Source: CAD feature listing. Evaluate the final solid. Frame: model axes, mm. A direction names the side the tool comes from. Round coordinates to 2 decimals unless told otherwise and drop trailing zeros. Order: outer loops, then holes, each group sorted by start corner. A loop starts at its lowest first (then second) coordinate and runs counter-clockwise, first axis right, second up. Notation, with made-up numbers: (-17.75, 29) - (32.25, 29) arc R19 ccw to (32.25, 45) - close; hole circle Ø10 at (-15, 17.5). An arc over 180 degrees is marked (long way). Put each result on its own line as item: value. Start each with the question number.
1) Line query: probe 1 along X at (y, z) = (0, 6.45); probe 2 along Y at (x, z) = (0, -21.65). Output: solid intervals per line, ascending. Write a range as [from, to].
2) Access query for faces 1 (the face through (-4.74, 2.79, 4.89)), 2 (the face through (0, 0, 5.8)), 3 (the face through (0, 0, 10.6)). Directions: +Z, -Z, +X, -X, +Y, -Y. A direction counts if a zero-diameter tool reaches every point of the face in a straight line with its end or side. Return the directions, or none.
3) Section C-C on z = 1. Output: boundary loops of the cut face in (x, y).
4) Section A-A on z = -21. Output: boundary loops of the cut face in (x, y), then the cut area to 3 significant figures.
5) Section D-D on y = -4.5. Output: boundary loops of the cut face in (x, z), then the cut area to 3 significant figures.
6) Contact query for flat-ended pins moving along their axis: P1, Ø2.5, axis at x = 0, y = 0, coming from the -Z side; P2, Ø5, axis at y = 3, z = -11.5, coming from the +X side; P3, Ø8, axis at x = 4.5, z = -7, coming from the +Y side; P4, Ø3.5, axis at x = 0.5, y = 0.5, coming from the +Z side. Output: stop coordinate, or through.
7) Section B-B on x = -5.5. Output: boundary loops of the cut face in (y, z), then the cut area to 3 significant figures.
8) Mould query, pull axis X, two halves, no side actions, for faces 4 (the face through (0, -5.5, 5)), 5 (the face through (0, 0, 7.3)), 6 (the face through (1.062, -4.783, -9.86)), 7 (the face through (-1.825, -1.4, 6.54)). Classes: +X half, -X half, draft (parallel to the pull), parting line (faces both ways), or undercut.
```python
from build123d import *

# Parameters (mm, degrees)
BOSS_EXTRUDE1_DEPTH = 4
BOSS_EXTRUDE2_DEPTH = 1.8
SKETCH3_R           = 2.65
SKETCH3_R_2         = 2.3
BOSS_EXTRUDE3_DEPTH = 5.8
BOSS_EXTRUDE4_START = -1
SKETCH4_R           = 3.15
BOSS_EXTRUDE4_DEPTH = 3.3
SKETCH5_R           = 4.9
BOSS_EXTRUDE5_DEPTH = 20
SKETCH6_R           = 3.15
SKETCH6_R_2         = 2.25
BOSS_EXTRUDE6_DEPTH = 6


with BuildPart() as part:
    # Sketch1 → Boss-Extrude1 (new body)
    with BuildSketch(Plane.XY):
        Polygon((8.082903769, 0), (4.041451884, 7), (-4.041451884, 7), (-8.082903769, 0), (-4.041451884, -7), (4.041451884, -7), align=None)
    extrude(amount=BOSS_EXTRUDE1_DEPTH)

    # Sketch2 → Boss-Extrude2 (add)
    with BuildSketch(Plane.XY.offset(4)):
        Polygon((6.350852961, 0), (3.175426481, 5.5), (-3.175426481, 5.5), (-6.350852961, 0), (-3.175426481, -5.5), (3.175426481, -5.5), align=None)
    extrude(amount=BOSS_EXTRUDE2_DEPTH)

    # Sketch3 → Boss-Extrude3 (add)
    with BuildSketch(Plane.XY.offset(5.8)):
        Circle(SKETCH3_R)
        Circle(SKETCH3_R_2, mode=Mode.SUBTRACT)
    extrude(amount=BOSS_EXTRUDE3_DEPTH)

    # Sketch4 → Boss-Extrude4 (add)
    with BuildSketch(Plane.XY.offset(11.6).offset(BOSS_EXTRUDE4_START)):
        Circle(SKETCH4_R)
    extrude(amount=-BOSS_EXTRUDE4_DEPTH)

    # Sketch5 → Boss-Extrude5 (add)
    with BuildSketch(Plane(origin=(0, 0, 0), x_dir=(-1, 0, 0), z_dir=(0, 0, -1))):
        Circle(SKETCH5_R)
    extrude(amount=BOSS_EXTRUDE5_DEPTH)

    # Sketch6 → Boss-Extrude6 (add)
    with BuildSketch(Plane(origin=(0, 0, -20), x_dir=(-1, 0, 0), z_dir=(0, 0, -1))):
        with Locations(Location((0, 0, 0), (0, 0, 180))):
            Circle(SKETCH6_R)
        Circle(SKETCH6_R_2, mode=Mode.SUBTRACT)
    extrude(amount=BOSS_EXTRUDE6_DEPTH)


solid = part.part
```
Answer sheet:
1. probe 1: [-2.65, -2.3], [2.3, 2.65]
1. probe 2: [-3.15, -2.25], [2.25, 3.15]
2. face 1: +Z, -X, +Y
2. face 2: none
2. face 3: +Z
3. outline: (-8.08, 0) - (-4.04, -7) - (4.04, -7) - (8.08, 0) - (4.04, 7) - (-4.04, 7) - close
4. outline: circle Ø6.3 at (0, 0); hole circle Ø4.5 at (0, 0)
4. area: 15.3 mm^2
5. outline: (-5.48, 0) - (-1.94, 0) - (-1.94, -20) - (1.94, -20) - (1.94, 0) - (5.48, 0) - (5.48, 4) - (3.75, 4) - (3.75, 5.8) - (-3.75, 5.8) - (-3.75, 4) - (-5.48, 4) - close
5. area: 135 mm^2
6. P1: z = -20
6. P2: x = 4.87
6. P3: y = 4.87
6. P4: z = 11.6
7. outline: (-4.47, 0) - (4.47, 0) - (4.47, 4) - (1.47, 4) - (1.47, 5.8) - (-1.47, 5.8) - (-1.47, 4) - (-4.47, 4) - close
7. area: 41.1 mm^2
8. face 4: draft
8. face 5: undercut
8. face 6: parting line
8. face 7: undercut
